Verification items for this drawing (mm, ordinates from the low corner). A direction names the side the tool comes from. Give positions to 0.01 mm unless a question says otherwise; leave off trailing zeros. Loops run counter-clockwise (first coordinate to the right, second up) from the corner with the lowest first, then second, coordinate; pieces in that order, holes last. Notation, with made-up numbers: (-39, -40) -> (0, -40) arc R23 cw to (0, -20) -> close; hole circle Ø9 at (-32, 87.5). An arc over 180 degrees is marked (long way). Answer as a JSON object with one key per item and string values.
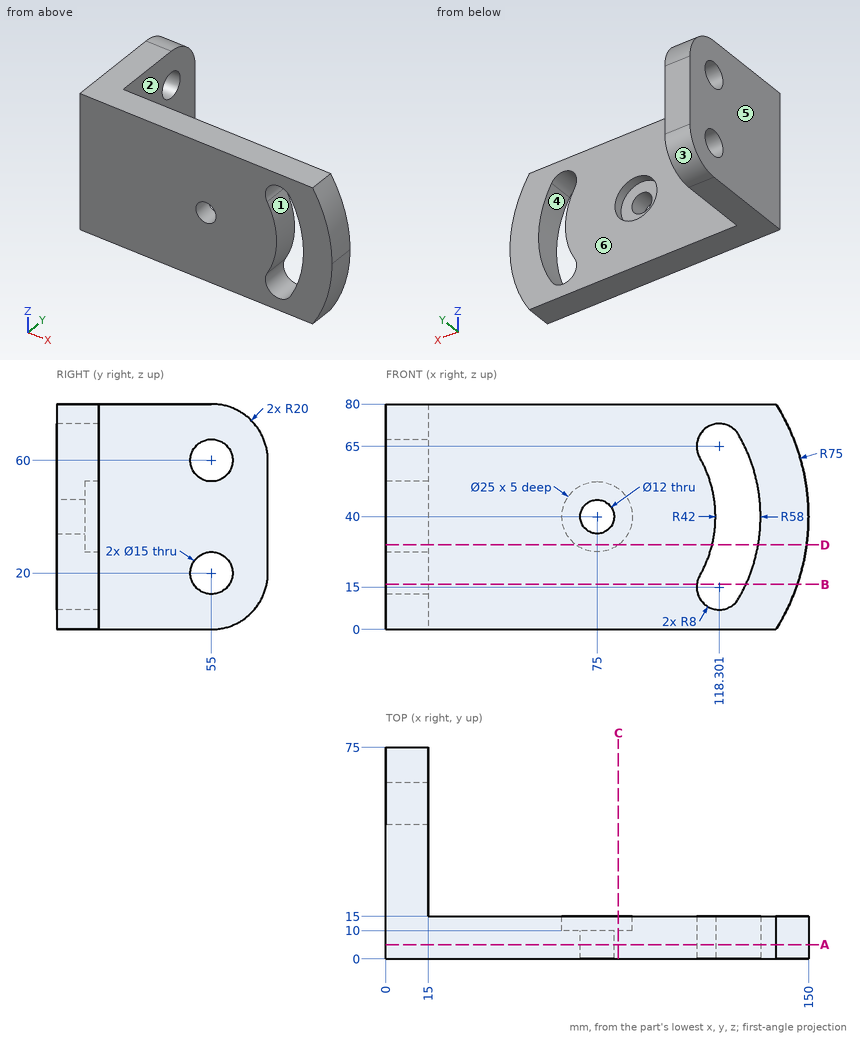
1) Section check B-B on z = 16. Record the cut outline in (x, y), plus the area to 3 significant figures.
Geometry check:
{"outline": "(0, 0) -> (110.36, 0) -> (110.36, 15) -> (15, 15) -> (15, 48.66) -> (0, 48.66) -> close; (0, 61.34) -> (15, 61.34) -> (15, 74.6) -> (0, 74.6) -> close; (127.8, 0) -> (146.06, 0) -> (146.06, 15) -> (127.8, 15) -> close", "area": "2,630 mm2"}
2) Material ranges on line 1 along Y through (x, z) = (122, 3), recorded low to high. Write a range as from..to.
Geometry check:
{"line 1": "y = 0..15"}
3) Section check A-A on y = 5. Record the cut outline in (x, z).
Geometry check:
{"outline": "(0, 0) -> (138.44, 0) arc R75 ccw to (138.44, 80) -> (0, 80) -> close; hole circle Ø12 at (75, 40); hole (111.37, 19) arc R8 ccw to (125.23, 11) arc R58 ccw to (125.23, 69) arc R8 ccw to (111.37, 61) arc R42 cw to start"}
4) Section check D-D on z = 30. Record the cut outline in (x, y).
Geometry check:
{"outline": "(0, 0) -> (115.79, 0) -> (115.79, 15) -> (82.5, 15) -> (82.5, 10) -> (67.5, 10) -> (67.5, 15) -> (15, 15) -> (15, 75) -> (0, 75) -> close; (132.13, 0) -> (149.33, 0) -> (149.33, 15) -> (132.13, 15) -> close"}
5) Tool access check on the marked faces 5 and 6. Record the directions out of +Z, -Z, +X, -X, +Y, -Y that give a thin tool (end or side, any length) a straight path to the whole face; none if there is none.
Geometry check:
{"face 5": "+Z, -Z, -X, +Y, -Y", "face 6": "+Z, -Z, +X, +Y"}
6) Depth check by flat-ended pin: P1, Ø4, axis at y = 61.5, z = 58, coming from the +X side; P2, Ø3, axis at y = 13, z = 54, coming from the +X side; P3, Ø7, axis at x = 75, z = 40, coming from the +Y side; P4, Ø1.5, axis at y = 14, z = 11.5, coming from the +X side. Enter the tip coordinate at first touch or a pass-through.
Geometry check:
{"P1": "stops at x = 15", "P2": "stops at x = 148.95", "P3": "passes through", "P4": "stops at x = 144.68"}
7) Section check C-C on x = 82.5. Record the cut outline in (y, z), plus the area to 3 significant figures.
Geometry check:
{"outline": "(0, 0) -> (15, 0) -> (15, 30) -> (10, 30) -> (10, 50) -> (15, 50) -> (15, 80) -> (0, 80) -> close", "area": "1,100 mm2"}
8) Draft check along X on the marked faces 1, 2, 3 and 4. Enter one of: pulls with the +X half, pulls with the -X half, needs draft (parallel to the pull), parting line crosses it, or undercut.
Geometry check:
{"face 1": "undercut", "face 2": "pulls with the +X half", "face 3": "needs draft", "face 4": "undercut"}
